from build123d import *

# Parameters (mm, degrees)
SKETCH1_W             = 200
SKETCH1_H             = 150
BOSS_EXTRUDE1_DEPTH   = 20
SKETCH2_R             = 3
BOSS_EXTRUDE2_DEPTH   = 5
M6_TAPPED_HOLE1_D     = 5
M6_TAPPED_HOLE1_DEPTH = 25
M6_TAPPED_HOLE1_TIP   = 1.502151548
CUT_EXTRUDE1_DEPTH    = 15
SKETCH6_W             = 16
SKETCH6_H             = 15
CUT_EXTRUDE2_DEPTH    = 129.937969582
FILLET1_R             = 2
M4_TAPPED_HOLE1_D     = 3.3
M4_TAPPED_HOLE1_DEPTH = 30
M4_TAPPED_HOLE1_TIP   = 0.991420021
FILLET2_R             = 10
M4_TAPPED_HOLE2_D     = 3.3
M4_TAPPED_HOLE2_DEPTH = 30
M4_TAPPED_HOLE2_TIP   = 0.991420021
CUT_EXTRUDE3_DEPTH    = 130.614813968
FILLET3_R             = 2


with BuildPart() as part:
    # Sketch1 → Boss-Extrude1 (new body)
    with BuildSketch(Plane(origin=(0, 0, 0), x_dir=(1, 0, 0), z_dir=(0, 1, 0))):
        Rectangle(SKETCH1_W, SKETCH1_H)
    extrude(amount=BOSS_EXTRUDE1_DEPTH)

    # Sketch2 → Boss-Extrude2 (add)
    with BuildSketch(Plane(origin=(0, 0, -75), x_dir=(-1, 0, 0), z_dir=(0, 0, -1))):
        with Locations(Location((0, 5, 0), (0, 0, 180))):
            Circle(SKETCH2_R)
    extrude(amount=BOSS_EXTRUDE2_DEPTH)

    # M6 Tapped Hole1
    with Locations(Plane(origin=(0, 0, -75), x_dir=(-1, 0, 0), z_dir=(0, 0, -1))):
        with Locations((0, 14)):
            Hole(M6_TAPPED_HOLE1_D / 2, depth=M6_TAPPED_HOLE1_DEPTH)
            with Locations((0, 0, -(M6_TAPPED_HOLE1_DEPTH + M6_TAPPED_HOLE1_TIP / 2))):  # 118° drill point
                Cone(0, M6_TAPPED_HOLE1_D / 2, M6_TAPPED_HOLE1_TIP, mode=Mode.SUBTRACT)

    # Sketch5 → Cut-Extrude1 (cut)
    with BuildSketch(Plane(origin=(0, 20, 0), x_dir=(1, 0, 0), z_dir=(0, 1, 0))):
        Polygon((-82.5, 50), (44.5, 50), (76.5, 50), (82.5, 50), (82.5, -30), (76.5, -30), (76.5, -51.78814737), (68.5, -51.78814737), (68.5, -66.78814737), (52.5, -66.78814737), (52.5, -51.78814737), (44.5, -51.78814737), (44.5, -30), (-82.5, -30), align=None)
    extrude(amount=-CUT_EXTRUDE1_DEPTH, mode=Mode.SUBTRACT)

    # Sketch6 → Cut-Extrude2 (cut, through all)
    with BuildSketch(Plane(origin=(0, 5, 0), x_dir=(1, 0, 0), z_dir=(0, 1, 0))):
        with Locations((60.5, -59.28814737)):
            Rectangle(SKETCH6_W, SKETCH6_H)
    extrude(amount=-CUT_EXTRUDE2_DEPTH, mode=Mode.SUBTRACT)

    # Fillet1
    fillet1_edges = [part.edges().sort_by_distance(p)[0] for p in [
        (-82.5, 12.5, -50),
        (-82.5, 12.5, 30),
        (82.5, 12.5, -50),
        (82.5, 12.5, 30),
        (76.5, 12.5, 30),
        (68.5, 12.5, 51.78814737),
        (68.5, 10, 66.78814737),
        (52.5, 10, 66.78814737),
        (52.5, 12.5, 51.78814737),
        (44.5, 12.5, 30),
    ]]
    fillet(fillet1_edges, radius=FILLET1_R)

    # M4 Tapped Hole1
    with Locations(Plane.ZY.offset(100)):
        with Locations((-5, 12)):
            Hole(M4_TAPPED_HOLE1_D / 2, depth=M4_TAPPED_HOLE1_DEPTH)
            with Locations((0, 0, -(M4_TAPPED_HOLE1_DEPTH + M4_TAPPED_HOLE1_TIP / 2))):  # 118° drill point
                Cone(0, M4_TAPPED_HOLE1_D / 2, M4_TAPPED_HOLE1_TIP, mode=Mode.SUBTRACT)

    # Fillet2
    fillet2_edges = [part.edges().sort_by_distance(p)[0] for p in [
        (100, 10, 75),
        (-100, 10, 75),
        (-100, 10, -75),
        (100, 10, -75),
    ]]
    fillet(fillet2_edges, radius=FILLET2_R)

    # M4 Tapped Hole2
    with Locations(Plane(origin=(0, 0, -75), x_dir=(-1, 0, 0), z_dir=(0, 0, -1))):
        with Locations((60, 12)):
            Hole(M4_TAPPED_HOLE2_D / 2, depth=M4_TAPPED_HOLE2_DEPTH)
            with Locations((0, 0, -(M4_TAPPED_HOLE2_DEPTH + M4_TAPPED_HOLE2_TIP / 2))):  # 118° drill point
                Cone(0, M4_TAPPED_HOLE2_D / 2, M4_TAPPED_HOLE2_TIP, mode=Mode.SUBTRACT)

    # Sketch13 → Cut-Extrude3 (cut, through all)
    with BuildSketch(Plane(origin=(0, 20, 0), x_dir=(1, 0, 0), z_dir=(0, 1, 0))):
        Polygon((73.5, -51.78814737), (115.827704394, -51.78814737), (115.827704394, -85.085952347), (72.5, -85.085952347), (-109.048113532, -107.181271315), (-117.406351495, -51.78814737), align=None)
    extrude(amount=-CUT_EXTRUDE3_DEPTH, mode=Mode.SUBTRACT)

    # Fillet3
    fillet3_edges = [part.edges().sort_by_distance(p)[0] for p in [
        (76.5, 12.5, 51.78814737),
        (44.5, 12.5, 51.78814737),
    ]]
    fillet(fillet3_edges, radius=FILLET3_R)


solid = part.part
Geometry check sheet. Reference: the model listing, model coordinates, mm. A direction names the side the tool comes from. Round coordinates to 2 decimals unless told otherwise and drop trailing zeros. Order: outer loops, then holes, each group sorted by start corner. A loop starts at its lowest first (then second) coordinate and runs counter-clockwise, first axis right, second up. Notation, with made-up numbers: (85, 7) -> (91, 7) arc R22 cw to (91, 32) -> close; hole circle Ø6 at (-9.5, 65). An arc over 180 degrees is marked (long way). Use one line per item in the form item = value.
1. Go/stop test with flat-tipped pins: pin 1 (4 mm diameter, centred on x = -10, z = 3, fed in from -Y); pin 2 (7.5 mm diameter, centred on x = -35.5, y = 11, fed in from -Z); pin 3 (1 mm diameter, centred on x = 25, z = -7.5, fed in from +Y). Record where each tip stops, or that it passes through.
Working result:
pin_1 = 0
pin_2 = -75
pin_3 = 5
2. Cross-section at B-B, the plane z = -35.5. Enter the section's corners in (x, y), plus the area to 4 significant figures.
Working result:
outline = (-100, 0) -> (100, 0) -> (100, 20) -> (82.5, 20) -> (82.5, 5) -> (-82.5, 5) -> (-82.5, 20) -> (-100, 20) -> close
area = 1,525 mm^2
3. Mould release check, pull along Z, two halves, no side actions. Record for faces 6 (the face through (-97.15, 10.14, -71.99)), 7 (the face through (44.5, 13, 41)), 8 (the face through (1, 11, -50)): pulls with the +Z half, pulls with the -Z half, needs draft (parallel to the pull), parting line crosses it, or undercut.
Working result:
face_6 = pulls with the -Z half
face_7 = needs draft
face_8 = undercut
4. Set-up check for faces 1 (the face through (0, 2, -77)), 2 (the face through (76.5, 13, 41)), 3 (the face through (-21, 10, 51.788)), 4 (the face through (-100, 10, -6)), 5 (the face through (-18, 13, 30)): record each of +Z, -Z, +X, -X, +Y, -Y from which the full face is reachable in a straight line by a thin tool's end or side.
Working result:
face_1 = -Z
face_2 = +Z, +Y
face_3 = +Z, +X, -X, +Y, -Y
face_4 = +Z, -Z, -X, +Y, -Y
face_5 = +Y
5. Scan lines: line 1 along X through (y, z) = (15.5, -3); line 2 along Z through (x, y) = (32.5, 12.25); line 3 along Y through (x, z) = (0, -62). Record each from-to range of solid material in increasing order. Write a range as from..to.
Working result:
line_1 = -100..-82.5, 82.5..100
line_2 = -75..-50, 30..51.79
line_3 = 0..11.5, 16.5..20
6. Cross-section at A-A, the plane x = -28. Enter the section's corners in (y, z), plus the area to 3 significant figures.
Working result:
outline = (0, -75) -> (20, -75) -> (20, -50) -> (5, -50) -> (5, 30) -> (20, 30) -> (20, 51.79) -> (0, 51.79) -> close
area = 1,340 mm^2
